```python
from build123d import *
from build123d.topology import SkipClean

# Parameters (mm, degrees)
BASE_AND_HUB_BODY_DEPTH       = 28
FRONT_START                   = 5
FRONT_HUB_BOSS_SKETCH_R       = 25
FRONT_HUB_BOSS_50_DEPTH       = 5
REAR_HUB_BOSS_SKETCH_R        = 25
REAR_HUB_BOSS_50_DEPTH        = 5
BEARING_BORE_SKETCH_R         = 12.5
BEARING_BORE_25_DEPTH         = 188.888264668
HUB_SLOT_SKETCH_R             = 8
HUB_SLOT_CUT_DEPTH            = 175.180940404
BASE_SLOT_SKETCH_R            = 8
BASE_SLOT_CUT_DEPTH           = 172.668284782
FLANGE_ARM_DEPTH              = 17
ARM_WEB_DEPTH                 = 22
WEB_RELIEF_CUT_DEPTH          = 5
FLANGE_RIM_DEPTH              = 5
ARM_FOOT_FILL_DEPTH           = 17
ARM_INFILL_DEPTH              = 17
FLANGE_BOLT_HOLES_SKETCH_R    = 6
FLANGE_BOLT_HOLES_4X_12_DEPTH = 218.917293143


with BuildPart() as part:
    # Base and Hub Profile Sketch → Base and Hub Body (new, symmetric)
    with BuildSketch(Plane.XY):
        with BuildLine():
            Line((0, 0), (165, 0))
            Line((165, 0), (165, 27))
            Line((165, 27), (104.732137495, 27))
            ThreePointArc((104.732137495, 27), (100.968274231, 28.708597057), (99.776781246, 32.666666667))
            ThreePointArc((99.776781246, 32.666666667), (76.670399482, 60.944132889), (50, 36))
            Line((50, 36), (50, 21))
            ThreePointArc((50, 21), (48.535533906, 17.464466094), (45, 16))
            Line((45, 16), (0, 16))
            Line((0, 16), (0, 0))
        make_face()
    extrude(amount=BASE_AND_HUB_BODY_DEPTH, both=True)

    # Front Hub Boss Sketch → Front Hub Boss Ø50 (add)
    with BuildSketch(Plane.XY.offset(28).offset(FRONT_START)):
        with Locations(Location((75, 36, 0), (0, 0, 180))):
            Circle(FRONT_HUB_BOSS_SKETCH_R)
    extrude(amount=-FRONT_HUB_BOSS_50_DEPTH)

    # Rear Hub Boss Sketch → Rear Hub Boss Ø50 (add)
    with SkipClean():  # the faces are left unmerged after this step: merging them gives an invalid solid
        with BuildSketch(Plane(origin=(0, 0, -28), x_dir=(-1, 0, 0), z_dir=(0, 0, -1))):
            with Locations((-75, 36)):
                Circle(REAR_HUB_BOSS_SKETCH_R)
        extrude(amount=REAR_HUB_BOSS_50_DEPTH)

    # Bearing Bore Sketch → Bearing Bore Ø25 (cut, through all)
    with SkipClean():  # the faces are left unmerged after this step: merging them gives an invalid solid
        with BuildSketch(Plane.XY.offset(33)):
            with Locations((75, 36)):
                Circle(BEARING_BORE_SKETCH_R)
        extrude(amount=-BEARING_BORE_25_DEPTH, mode=Mode.SUBTRACT)

    # Hub Slot Sketch → Hub Slot Cut (cut, through all)
    with SkipClean():  # the faces are left unmerged after this step: merging them gives an invalid solid
        with BuildSketch(Plane(origin=(0, 16, 0), x_dir=(1, 0, 0), z_dir=(0, 1, 0))):
            with Locations(Location((25, 3, 0), (0, 0, 270))):
                Circle(HUB_SLOT_SKETCH_R)
        extrude(amount=-HUB_SLOT_CUT_DEPTH, mode=Mode.SUBTRACT)

    # Base Slot Sketch → Base Slot Cut (cut, through all)
    with SkipClean():  # the faces are left unmerged after this step: merging them gives an invalid solid
        with BuildSketch(Plane(origin=(0, 27, 0), x_dir=(1, 0, 0), z_dir=(0, 1, 0))):
            with Locations(Location((140, 3, 0), (0, 0, 180))):
                Circle(BASE_SLOT_SKETCH_R)
        extrude(amount=-BASE_SLOT_CUT_DEPTH, mode=Mode.SUBTRACT)

    # Flange Arm Sketch → Flange Arm (add)
    with SkipClean():  # the faces are left unmerged after this step: merging them gives an invalid solid
        with BuildSketch(Plane.XY.offset(28)):
            with BuildLine():
                ThreePointArc((164.887685495, 35.975383738), (138.674843146, 99.614923148), (75.157577255, 126.122676998))
                ThreePointArc((75.157577255, 126.122676998), (60.112682879, 111.167706145), (75.067653733, 96.122811769))
                ThreePointArc((75.067653733, 96.122811769), (117.41249766, 78.450975869), (134.887725893, 36.024616262))
                ThreePointArc((134.887725893, 36.024616262), (149.863089432, 21.000020199), (164.887685495, 35.975383738))
            make_face()
        extrude(amount=-FLANGE_ARM_DEPTH)

    # Arm Web Sketch → Arm Web (add)
    with SkipClean():  # the faces are left unmerged after this step: merging them gives an invalid solid
        with BuildSketch(Plane.XY.offset(33)):
            with BuildLine():
                Line((90.112682879, 111.167706145), (60.112682879, 111.167706145))
                Line((60.112682879, 111.167706145), (60.112682879, 56.084018247))
                ThreePointArc((60.112682879, 56.084018247), (75.140854857, 60.999603195), (90.112682879, 55.914989736))
                Line((90.112682879, 55.914989736), (90.112682879, 111.167706145))
            make_face()
        extrude(amount=-ARM_WEB_DEPTH)

    # Web Relief Sketch → Web Relief Cut (cut)
    with SkipClean():  # the faces are left unmerged after this step: merging them gives an invalid solid
        with BuildSketch(Plane.XY.offset(33)):
            with BuildLine():
                Line((60.112682879, 56.084018247), (60.112682879, 112.084018247))
                Line((60.112682879, 112.084018247), (90.112682879, 112.084018247))
                Line((90.112682879, 112.084018247), (90.112682879, 55.914989736))
                ThreePointArc((90.112682879, 55.914989736), (75.140854857, 60.999603195), (60.112682879, 56.084018247))
            make_face()
        extrude(amount=-WEB_RELIEF_CUT_DEPTH, mode=Mode.SUBTRACT)

    # Flange Rim Sketch → Flange Rim (add)
    with SkipClean():  # the faces are left unmerged after this step: merging them gives an invalid solid
        with BuildSketch(Plane.XY.offset(28)):
            with BuildLine():
                ThreePointArc((164.935672679, 39.402172812), (137.425172995, 100.831302444), (75, 126))
                ThreePointArc((75, 126), (60, 111), (75, 96))
                ThreePointArc((75, 96), (116.616781997, 79.220868296), (134.957115119, 38.268115208))
                ThreePointArc((134.957115119, 38.268115208), (150.513422701, 23.84586523), (164.935672679, 39.402172812))
            make_face()
        extrude(amount=FLANGE_RIM_DEPTH)

    # Arm Foot Fill Sketch → Arm Foot Fill (add)
    with SkipClean():  # the faces are left unmerged after this step: merging them gives an invalid solid
        with BuildSketch(Plane.XY.offset(28)):
            with BuildLine():
                ThreePointArc((135.089588319, 33.547303087), (134.158093135, 29.984243626), (132, 27))
                Line((132, 27), (137.819213879, 27))
                ThreePointArc((137.819213879, 27), (137.363665204, 27.696139518), (136.94629296, 28.415816692))
                ThreePointArc((136.94629296, 28.415816692), (135.782620766, 30.896415066), (135.089588319, 33.547303087))
            make_face()
        extrude(amount=-ARM_FOOT_FILL_DEPTH)

    # Arm Infill Sketch → Arm Infill (add)
    with SkipClean():  # the faces are left unmerged after this step: merging them gives an invalid solid
        with BuildSketch(Plane.XY.offset(28)):
            with BuildLine():
                Line((161.887705694, 27), (165, 27))
                Line((165, 27), (164.887685495, 35.975383738))
                ThreePointArc((164.887685495, 35.975383738), (164.1140582, 31.244908584), (161.887705694, 27))
            make_face()
        extrude(amount=-ARM_INFILL_DEPTH)

    # Flange Bolt Holes Sketch → Flange Bolt Holes 4xØ12 (cut, through all)
    with SkipClean():  # the faces are left unmerged after this step: merging them gives an invalid solid
        with BuildSketch(Plane.XY.offset(33)):
            with Locations((150, 36)):
                Circle(FLANGE_BOLT_HOLES_SKETCH_R)
            with Locations((75, 111)):
                Circle(FLANGE_BOLT_HOLES_SKETCH_R)
            with Locations((112.5, 100.951905284)):
                Circle(FLANGE_BOLT_HOLES_SKETCH_R)
            with Locations((139.951905284, 73.5)):
                Circle(FLANGE_BOLT_HOLES_SKETCH_R)
        extrude(amount=-FLANGE_BOLT_HOLES_4X_12_DEPTH, mode=Mode.SUBTRACT)


solid = part.part
```
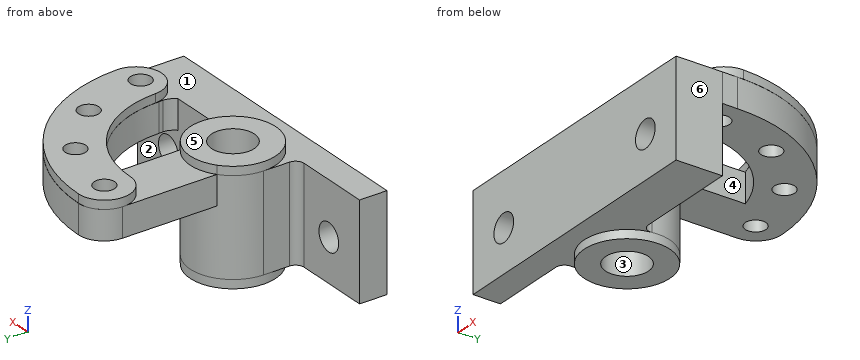
For this review, take the finished solid that the model builds, in its own axes (mm). Face numbers are marked on the shaded views. A direction names the side the tool comes from. Round coordinates to 2 decimals unless told otherwise and drop trailing zeros. Write each loop counter-clockwise with the first axis right and the second up, starting at its lowest first coordinate (ties: lowest second). Pieces come first, ordered by that corner, then holes. Notation, with made-up numbers: (-12, 17.25) - (6, 17.25) arc R34 ccw to (6, 53.25) - close; hole circle Ø11 at (76, 64.25). An arc over 180 degrees is marked (long way). Answer as a JSON object with one key per item and string values.
1. We need section A-A on x = 25. Give the boundary of the cut face in (y, z).
Response values:
{"outline": "(0, -28) - (16, -28) - (16, -11) - (0, -11) - close; (0, 5) - (16, 5) - (16, 28) - (0, 28) - close"}
2. We need section C-C on z = -3. Give the boundary of the cut face in (x, y).
Response values:
{"outline": "(0, 0) - (17, 0) - (17, 16) - (0, 16) - close; (33, 0) - (132, 0) - (132, 27) - (104.73, 27) arc R5 cw to (99.78, 32.67) arc R25 ccw (long way) to (50, 36) - (50, 21) arc R5 cw to (45, 16) - (33, 16) - close; (148, 0) - (165, 0) - (165, 27) - (148, 27) - close; hole circle Ø25 at (75, 36)"}
3. Tool access review of the marked faces 1 and 2: name each direction out of +Z, -Z, +X, -X, +Y, -Y from which nothing blocks a thin tool from reaching the whole face with its end or side.
Response values:
{"face 1": "+Z, -Y", "face 2": "-Z"}
4. For pin 1 Ø18.5 at (y, z) = (74, 16.5) entering from +X; pin 2 Ø2 at (y, z) = (48.5, 4.5) entering from -X; pin 3 Ø12 at (x, y) = (64, 60.5) entering from +Z; pin 4 Ø18.5 at (y, z) = (89, 21) entering from -X, all flat-tipped, find the tip position at first contact; note any pin that passes through.
Response values:
{"pin 1": "stops at x = 160.21", "pin 2": "stops at x = 52.8", "pin 3": "stops at z = 33", "pin 4": "stops at x = 60.11"}
5. We need section B-B on y = 73.5. Count the separate pieces of the cut face and the enclosed holes in it, then the cut area to 3 significant figures.
Response values:
{"separate pieces": "3", "enclosed holes": "0", "area": "1,010 mm2"}
6. Draft analysis for pull direction X (two halves, no side actions). For the marked faces 3, 4, 5 and 6, state which applies: +X half, -X half, draft (parallel to the pull), parting line (faces both ways), or undercut.
Response values:
{"face 3": "undercut", "face 4": "undercut", "face 5": "draft", "face 6": "+X half"}
7. To check wall thickness, follow line 1 along X through (y, z) = (8, -2.5); line 2 along Y through (x, z) = (75, 17); line 3 along Y through (x, z) = (112.5, 18). State the ranges of each line that lie inside material, in increasing order.
Response values:
{"line 1": "x = 0 to 17.02, 32.98 to 132.02, 147.98 to 165", "line 2": "y = 0 to 23.5, 48.5 to 105, 117 to 126.12", "line 3": "y = 0 to 27, 82.87 to 94.95, 106.95 to 117.89"}
